Can you work these out from the model? Positions are in its coordinate system, mm. Give positions to 0.01 mm unless a question says otherwise; leave off trailing zeros. Order: outer loops, then holes, each group sorted by start corner. A loop starts at its lowest first (then second) coordinate and runs counter-clockwise, first axis right, second up. Notation, with made-up numbers: (15.25, 25.5) - (24.25, 25.5) arc R15 ccw to (24.25, 44.5) - close; hole circle Ø11 at (-6, 24). An arc over 180 degrees is marked (long way). Return JSON: item names as keys, results as strings.
```python
from build123d import *

# Parameters (mm, degrees)
EXTRUDE_1_DEPTH     = 10
SKETCH_2_R          = 6.25
CUT_EXTRUDE_1_DEPTH = 220.431082575
CHAMFER_1_SIZE      = 2
CHAMFER_2_SIZE      = 3.5


with BuildPart() as part:
    # 草图1 → 凸台-拉伸1 (new body)
    with BuildSketch(Plane.XY):
        with BuildLine():
            Line((-155, 0), (-99.5, 0))
            Line((-99.5, 0), (-99.5, 2.5))
            Line((-99.5, 2.5), (-99.5, 81.5))
            ThreePointArc((-99.5, 81.5), (-94.227922061, 94.227922061), (-81.5, 99.5))
            Line((-81.5, 99.5), (81.5, 99.5))
            ThreePointArc((81.5, 99.5), (94.227922061, 94.227922061), (99.5, 81.5))
            Line((99.5, 81.5), (99.5, 2.5))
            Line((99.5, 2.5), (99.5, 0))
            Line((99.5, 0), (155, 0))
            Line((155, 0), (155, 2.5))
            Line((155, 2.5), (155, 135))
            ThreePointArc((155, 135), (149.142135624, 149.142135624), (135, 155))
            Line((135, 155), (-135, 155))
            ThreePointArc((-135, 155), (-149.142135624, 149.142135624), (-155, 135))
            Line((-155, 135), (-155, 2.5))
            Line((-155, 2.5), (-155, 0))
        make_face()
    extrude(amount=EXTRUDE_1_DEPTH)

    # 草图2 → 切除-拉伸1 (cut, through all)
    with BuildSketch(Plane.XY.offset(10)):
        with Locations((0, 137)):
            Circle(SKETCH_2_R)
        with Locations((0, -137)):
            Circle(SKETCH_2_R)
        with Locations((-137, 137)):
            Circle(SKETCH_2_R)
        with Locations((137, 137)):
            Circle(SKETCH_2_R)
        with Locations((-137, -137)):
            Circle(SKETCH_2_R)
        with Locations((137, -137)):
            Circle(SKETCH_2_R)
        with Locations((-137, 15)):
            Circle(SKETCH_2_R)
        with Locations((-137, -15)):
            Circle(SKETCH_2_R)
        with Locations((137, -15)):
            Circle(SKETCH_2_R)
        with Locations(Location((137, 15, 0), (0, 0, 180))):
            Circle(SKETCH_2_R)
    extrude(amount=-CUT_EXTRUDE_1_DEPTH, mode=Mode.SUBTRACT)

    # 倒角1
    chamfer_1_edges = [part.edges().sort_by_distance(p)[0] for p in [
        (-99.5, 0, 5),
        (-155, 0, 5),
        (155, 0, 5),
        (99.5, 0, 5),
    ]]
    chamfer(chamfer_1_edges, length=CHAMFER_1_SIZE)

    # 倒角2
    chamfer_2_edges = [part.edges().sort_by_distance(p)[0] for p in [
        (99.5, 41.75, 0),
        (94.227922061, 94.227922061, 0),
        (0, 99.5, 0),
        (-94.227922061, 94.227922061, 0),
        (-99.5, 41.75, 0),
        (99.5, 41.75, 10),
        (94.227922061, 94.227922061, 10),
        (-99.5, 41.75, 10),
        (-94.227922061, 94.227922061, 10),
        (0, 99.5, 10),
    ]]
    chamfer(chamfer_2_edges, length=CHAMFER_2_SIZE)


solid = part.part
```
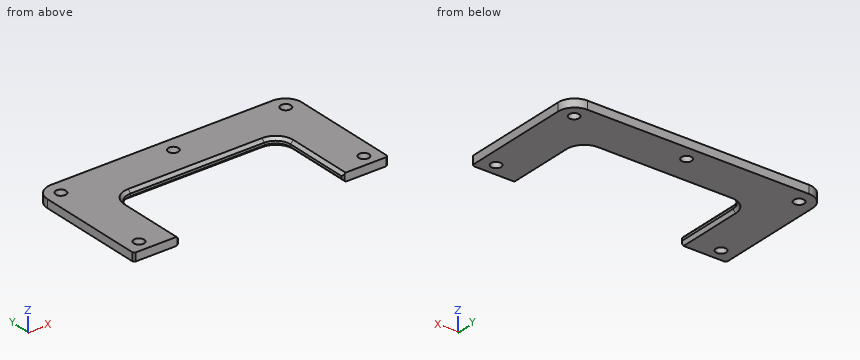
1. Suppose I cut it at B-B (y = 50). List the corners of the cut face in (x, z) for me, plus the area to 3 significant figures.
Checks:
{"outline": "(-155, 0) - (-103, 0) - (-99.5, 3.5) - (-99.5, 6.5) - (-103, 10) - (-155, 10) - close; (99.5, 3.5) - (103, 0) - (155, 0) - (155, 10) - (103, 10) - (99.5, 6.5) - close", "area": "1,090 mm^2"}
2. For pin 1 Ø4 at (x, z) = (70, 4.5) entering from -Y; pin 2 Ø5 at (x, z) = (86, 6) entering from -Y, each with a flat end and sliding along its axis, tell me the tip position at first contact or that it passes through.
Checks:
{"pin 1": "y = 99.5", "pin 2": "y = 98.08"}
3. If I drill on L1, parallel to Y at x = -137, z = 4.5; L2, parallel to Y at x = -132, z = 3.75; L3, parallel to X at y = 66.5, z = 8.25, over which ranges is the centre line in solid material (lowest first)? Write a range as [from, to].
Checks:
{"L1": "[0, 8.75], [21.25, 130.75], [143.25, 154.9]", "L2": "[0, 11.25], [18.75, 133.25], [140.75, 155]", "L3": "[-155, -101.25], [101.25, 155]"}
4. Suppose I cut it at A-A (x = 0). List the corners of the cut face in (y, z) for me, plus the area to 3 significant figures.
Checks:
{"outline": "(99.5, 3.5) - (103, 0) - (130.75, 0) - (130.75, 10) - (103, 10) - (99.5, 6.5) - close; (143.25, 0) - (155, 0) - (155, 10) - (143.25, 10) - close", "area": "418 mm^2"}
5. Suppose I cut it at C-C (y = 15). List the corners of the cut face in (x, z) for me, plus the area to 4 significant figures.
Checks:
{"outline": "(-155, 0) - (-143.25, 0) - (-143.25, 10) - (-155, 10) - close; (-130.75, 0) - (-103, 0) - (-99.5, 3.5) - (-99.5, 6.5) - (-103, 10) - (-130.75, 10) - close; (99.5, 3.5) - (103, 0) - (130.75, 0) - (130.75, 10) - (103, 10) - (99.5, 6.5) - close; (143.25, 0) - (155, 0) - (155, 10) - (143.25, 10) - close", "area": "835.5 mm^2"}
6. Suppose I cut it at D-D (x = 66). List the corners of the cut face in (y, z) for me.
Checks:
{"outline": "(99.5, 3.5) - (103, 0) - (155, 0) - (155, 10) - (103, 10) - (99.5, 6.5) - close"}
